from build123d import *

# Parameters (mm, degrees)
SKETCH_1_W                   = 36
SKETCH_1_H                   = 11
CUT_EXTRUDE_1_DEPTH          = 53.086466572
SKETCH_3_W                   = 21
SKETCH_3_H                   = 120
HOLE_WIZARD_M27_1_D          = 30
HOLE_WIZARD_M6_1_D           = 6.6
HOLE_WIZARD_M6_1_DEPTH       = 131
HOLE_WIZARD_M6_1_CBORE_D     = 11
HOLE_WIZARD_M6_1_CBORE_DEPTH = 6.4
CHAMFER_1_SIZE               = 1


with BuildPart() as part:
    # 草图1 → 旋转1 (revolve)
    with BuildSketch(Plane.XZ, mode=Mode.PRIVATE) as revolve_1_sk:
        with Locations((18, 5.5)):
            Rectangle(SKETCH_1_W, SKETCH_1_H)
    revolve(revolve_1_sk.sketch.rotate(Axis((0, 0, 11), (0, 0, -1)), 180), axis=Axis((0, 0, 11), (0, 0, -1)))

    # 草图2 → 切除-拉伸1 (cut, through all)
    with BuildSketch(Plane.XY.offset(11)):
        with BuildLine():
            Line((20.02023451, 29.919729447), (16.263455967, 26.162950904))
            ThreePointArc((16.263455967, 26.162950904), (16.263455967, 16.263455967), (26.162950904, 16.263455967))
            Line((26.162950904, 16.263455967), (29.919729447, 20.02023451))
            ThreePointArc((29.919729447, 20.02023451), (25.455844123, 25.455844123), (20.02023451, 29.919729447))
        make_face()
    extrude(amount=-CUT_EXTRUDE_1_DEPTH, mode=Mode.SUBTRACT)

    # 草图3 → 旋转2 (revolve)
    with BuildSketch(Plane.XZ, mode=Mode.PRIVATE) as revolve_2_sk:
        with Locations((10.5, 71)):
            Rectangle(SKETCH_3_W, SKETCH_3_H)
    revolve(revolve_2_sk.sketch.rotate(Axis((0, 0, 131), (0, 0, -1)), 180), axis=Axis((0, 0, 131), (0, 0, -1)))

    # M27 间隙孔1 (through all)
    with Locations(Plane(origin=(0, 0, 0), x_dir=(-1, 0, 0), z_dir=(0, 0, -1))):
        with Locations((0, 0)):
            Hole(HOLE_WIZARD_M27_1_D / 2)

    # M6 六角头螺栓的柱形沉头孔1
    with Locations(Plane(origin=(0, 0, 0), x_dir=(-1, 0, 0), z_dir=(0, 0, -1))):
        with Locations((0, 27.5), (27.5, 0), (0, -27.5), (-27.5, 0)):
            CounterBoreHole(HOLE_WIZARD_M6_1_D / 2, HOLE_WIZARD_M6_1_CBORE_D / 2, HOLE_WIZARD_M6_1_CBORE_DEPTH, depth=HOLE_WIZARD_M6_1_DEPTH)

    # 倒角1
    chamfer_1_edges = [part.edges().sort_by_distance(p)[0] for p in [
        (-25.455844123, -25.455844123, 0),
        (21, 0, 131),
        (-15, 0, 0),
    ]]
    chamfer(chamfer_1_edges, length=CHAMFER_1_SIZE)


solid = part.part
Input: part model. Units: mm. Frame: model coordinates. A direction names the side the tool comes from. Round coordinates to 2 decimals unless told otherwise and drop trailing zeros. Loops run counter-clockwise (first coordinate to the right, second up) from the corner with the lowest first, then second, coordinate; pieces in that order, holes last. Notation, with made-up numbers: M -9.5,-37 L 10.5,-37 A17 cw 10.5,-33 Z; hole C 40,-16.5 d10. An arc over 180 degrees is marked long. Answer as CSV lines item,"result". Start each with the question number.
(1) Reachability of faces 4 (the cylindrical face through (-14.985, 0.66, 66.91)), 5 (the cylindrical face through (0.716, 32.953, 3.155)), 6 (the flat face through (28, 18.1, 5.6)) from +Z, -Z, +X, -X, +Y, -Y: full face, straight path, thin tool, end or side. Return the list, or none.
(2) Line query: line 1 (Y direction, x = 0, z = 9.6); line 2 (Y direction, x = 0, z = 3.5); line 3 (Z direction, x = -22.5, y = 24). Output: solid intervals per line, ascending. Write a range as [from, to].
(3) Section A-A, the plane x = 0. State how many separate pieces and enclosed holes the cut face has, plus the area to 3 significant figures.
(4) Section B-B, the plane z = 13. Output: boundary loops of the cut face in (x, y).
(5) Draft query along Y for faces 1 (the cylindrical face through (-20.03, 6.31, 71.33)), 2 (the flat face through (15, -15, 11)), 3 (the cylindrical face through (33, 0, 3)). Return one class per face: released by +Y, released by -Y, zero draft, split by the parting line, or undercut.
(6) First-contact query: pin 1 (7.5 mm diameter, centred on x = 0, y = 27.5, fed in from -Z); pin 2 (10 mm diameter, centred on x = -27.5, y = 0, fed in from +Z); pin 3 (6 mm diameter, centred on y = 12.5, z = 55.5, fed in from -X). Flat tips, straight axial feed; report the tip coordinate or a pass-through.
Values found:
1,face 4,"+Z, -Z"
1,face 5,"-Z"
1,face 6,"+Z, -Z, +Y"
2,line 1,"y = [-36, -30.8], [-24.2, -15], [15, 24.2], [30.8, 36]"
2,line 2,"y = [-36, -33], [-22, -15], [15, 22], [33, 36]"
2,line 3,"z = [0, 11]"
3,separate pieces,"4"
3,enclosed holes,"0"
3,area,"1,700 mm²"
4,outline,"C 0,0 d42; hole C 0,0 d30"
5,face 1,"split by the parting line"
5,face 2,"zero draft"
5,face 3,"undercut"
6,pin 1,"stops at z = 6.4"
6,pin 2,"stops at z = 11"
6,pin 3,"stops at x = -18.73"
